Geometry check sheet. Reference: the model listing, model coordinates, mm. Face numbers are marked on the shaded views. A direction names the side the tool comes from. Round coordinates to 2 decimals unless told otherwise and drop trailing zeros. Loops run counter-clockwise (first coordinate to the right, second up) from the corner with the lowest first, then second, coordinate; pieces in that order, holes last.
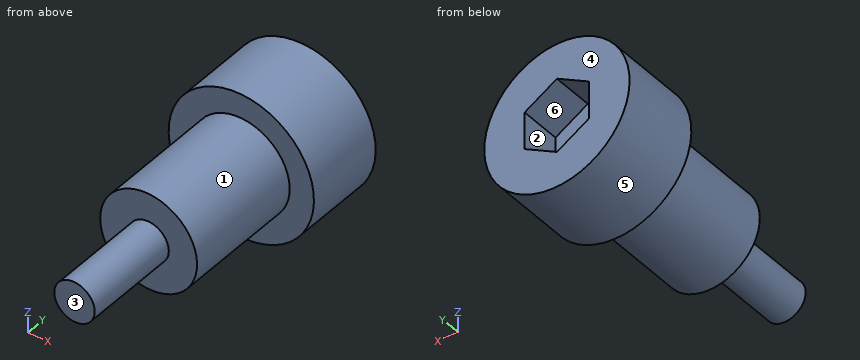
```python
from build123d import *

# Parameters (mm, degrees)
SKETCH1_R           = 2.5
BOSS_EXTRUDE1_DEPTH = 12
SKETCH2_R           = 6
BOSS_EXTRUDE2_DEPTH = 15
SKETCH3_R           = 9
BOSS_EXTRUDE3_DEPTH = 10
CUT_EXTRUDE1_DEPTH  = 5


with BuildPart() as part:
    # Sketch1 → Boss-Extrude1 (new body)
    with BuildSketch(Plane(origin=(0, 0, 0), x_dir=(1, 0, 0), z_dir=(0, 1, 0))):
        with Locations(Location((0, 0, 0), (0, 0, 270))):
            Circle(SKETCH1_R)
    extrude(amount=BOSS_EXTRUDE1_DEPTH)

    # Sketch2 → Boss-Extrude2 (add)
    with BuildSketch(Plane(origin=(0, 12, 0), x_dir=(1, 0, 0), z_dir=(0, 1, 0))):
        with Locations(Location((0, 0, 0), (0, 0, 270))):
            Circle(SKETCH2_R)
    extrude(amount=BOSS_EXTRUDE2_DEPTH)

    # Sketch3 → Boss-Extrude3 (add)
    with BuildSketch(Plane(origin=(0, 27, 0), x_dir=(1, 0, 0), z_dir=(0, 1, 0))):
        with Locations(Location((0, 0, 0), (0, 0, 270))):
            Circle(SKETCH3_R)
    extrude(amount=BOSS_EXTRUDE3_DEPTH)

    # Sketch4 → Cut-Extrude1 (cut)
    with BuildSketch(Plane(origin=(0, 37, 0), x_dir=(1, 0, 0), z_dir=(0, 1, 0))):
        Polygon((0, 4.618802154), (-4, 2.309401077), (-4, -2.309401077), (0, -4.618802154), (4, -2.309401077), (4, 2.309401077), align=None)
    extrude(amount=-CUT_EXTRUDE1_DEPTH, mode=Mode.SUBTRACT)


solid = part.part
```
1) Sectioned sample at A-A, the plane y = 35. Record the cut outline in (x, z), then the cut area to 3 significant figures.
Report:
outline: circle Ø18 at (0, 0); hole (-4, -2.31) - (0, -4.62) - (4, -2.31) - (4, 2.31) - (0, 4.62) - (-4, 2.31) - close
area: 199 mm2
2) Scan lines: line 1 along Y through (x, z) = (-2, 0.25); line 2 along Y through (x, z) = (-7, -1); line 3 along X through (y, z) = (32.5, -3.5). Record each from-to range of solid material in increasing order.
Report:
line 1: y = 0 to 32
line 2: y = 27 to 37
line 3: x = -8.29 to -1.94, 1.94 to 8.29
3) Gauge pin test, flat ends, axial feed: pin 1 (10 mm diameter, centred on y = 17.5, z = -6, fed in from +X); pin 2 (4 mm diameter, centred on x = 0, y = 22, fed in from -Z); pin 3 (4 mm diameter, centred on x = 0, z = -0.5, fed in from +Y). Record the tip position at first contact, or that the pin passes through.
Report:
pin 1: stops at x = 5.92
pin 2: stops at z = -6
pin 3: stops at y = 32
4) Mould release check, pull along Z, two halves, no side actions. Record for the marked faces 4, 5 and 6: +Z half, -Z half, draft (parallel to the pull), parting line (faces both ways), or undercut.
Report:
face 4: draft
face 5: parting line
face 6: undercut
5) Sectioned sample at D-D, the plane y = 15.5. Record the cut outline in (x, z), then the cut area to 3 significant figures.
Report:
outline: circle Ø12 at (0, 0)
area: 113 mm2
6) Sectioned sample at C-C, the plane x = -3.5. Record the cut outline in (y, z), then the cut area to 3 significant figures.
Report:
outline: (12, -4.87) - (27, -4.87) - (27, -8.29) - (37, -8.29) - (37, -2.6) - (32, -2.6) - (32, 2.6) - (37, 2.6) - (37, 8.29) - (27, 8.29) - (27, 4.87) - (12, 4.87) - close
area: 286 mm2
7) Sectioned sample at B-B, the plane z = 0. Record the cut outline in (x, y), then the cut area to 3 significant figures.
Report:
outline: (-9, 27) - (-6, 27) - (-6, 12) - (-2.5, 12) - (-2.5, 0) - (2.5, 0) - (2.5, 12) - (6, 12) - (6, 27) - (9, 27) - (9, 37) - (4, 37) - (4, 32) - (-4, 32) - (-4, 37) - (-9, 37) - close
area: 380 mm2
8) Access from +Z, -Z, +X, -X, +Y, -Y to the whole of each face (thin tool, end or side, straight path). Record for the marked faces 1, 2 and 3.
Report:
face 1: -Y
face 2: +Y
face 3: +Z, -Z, +X, -X, -Y
